```python
from build123d import *

# Parameters (mm, degrees)
SKETCH_1_W             = 49.2
SKETCH_1_H             = 40
EXTRUDE_1_DEPTH        = 8
HOLE_WIZARD_M4_1_D     = 3.3
HOLE_WIZARD_M4_1_DEPTH = 10.1
HOLE_WIZARD_M4_1_TIP   = 0.991420021
CHAMFER_1_SIZE         = 2
SKETCH_8_W             = 55.272888483
SKETCH_8_H             = 36.198084545
CUT_EXTRUDE_3_DEPTH    = 2
SKETCH_9_R             = 4.25
CUT_EXTRUDE_4_DEPTH    = 25
HOLE_WIZARD_M4_2_D     = 3.3
HOLE_WIZARD_M4_2_DEPTH = 10.1
HOLE_WIZARD_M4_2_TIP   = 0.991420021


with BuildPart() as part:
    # 草图1 → 凸台-拉伸1 (new body)
    with BuildSketch(Plane.XY):
        Rectangle(SKETCH_1_W, SKETCH_1_H)
    extrude(amount=EXTRUDE_1_DEPTH)

    # M4 螺纹孔1
    with Locations(Plane(origin=(0, -20, 0), x_dir=(-1, 0, 0), z_dir=(0, -1, 0))):
        with Locations((12.7, -4), (-12.7, -4)):
            Hole(HOLE_WIZARD_M4_1_D / 2, depth=HOLE_WIZARD_M4_1_DEPTH)
            with Locations((0, 0, -(HOLE_WIZARD_M4_1_DEPTH + HOLE_WIZARD_M4_1_TIP / 2))):  # 118° drill point
                Cone(0, HOLE_WIZARD_M4_1_D / 2, HOLE_WIZARD_M4_1_TIP, mode=Mode.SUBTRACT)

    # 倒角1
    chamfer_1_edges = [part.edges().sort_by_distance(p)[0] for p in [
        (-24.6, 20, 4),
        (24.6, 20, 4),
    ]]
    chamfer(chamfer_1_edges, length=CHAMFER_1_SIZE)

    # 草图8 → 切除-拉伸3 (cut)
    with BuildSketch(Plane.XY.offset(8)):
        with Locations((2.667874568, 4.099042273)):
            Rectangle(SKETCH_8_W, SKETCH_8_H)
    extrude(amount=-CUT_EXTRUDE_3_DEPTH, mode=Mode.SUBTRACT)

    # 草图9 → 切除-拉伸4 (cut)
    with BuildSketch(Plane(origin=(0, 0, 0), x_dir=(-1, 0, 0), z_dir=(0, 0, -1))):
        with Locations((-15, 6)):
            Circle(SKETCH_9_R)
        with Locations((15, 6)):
            Circle(SKETCH_9_R)
    extrude(amount=-CUT_EXTRUDE_4_DEPTH, mode=Mode.SUBTRACT)

    # M4 螺纹孔2
    with Locations(Plane.XY.offset(6)):
        with Locations((0, -4)):
            Hole(HOLE_WIZARD_M4_2_D / 2, depth=HOLE_WIZARD_M4_2_DEPTH)
            with Locations((0, 0, -(HOLE_WIZARD_M4_2_DEPTH + HOLE_WIZARD_M4_2_TIP / 2))):  # 118° drill point
                Cone(0, HOLE_WIZARD_M4_2_D / 2, HOLE_WIZARD_M4_2_TIP, mode=Mode.SUBTRACT)


solid = part.part
```
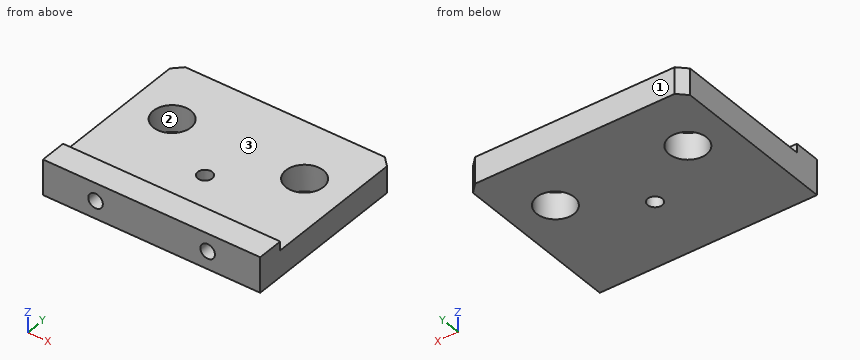
Can you work these out from the model? Positions are in its coordinate system, mm. Face numbers are marked on the shaded views. Coordinates: 2 decimals unless noted, no trailing zeros. Loops run counter-clockwise (first coordinate to the right, second up) from the corner with the lowest first, then second, coordinate; pieces in that order, holes last. Notation, with made-up numbers: (-39.75, 57) -> (-34.75, 57) arc R23 ccw to (-34.75, 87) -> close; hole circle Ø2 at (0.25, 13.5). An arc over 180 degrees is marked (long way). Answer as a JSON object with one key per item and string values.
1) Imagine slicing it at B-B (y = -4). Please give me the cut outline in (x, z).
Results:
{"outline": "(-24.6, 0) -> (-1.65, 0) -> (-1.65, 6) -> (-24.6, 6) -> close; (1.65, 0) -> (24.6, 0) -> (24.6, 6) -> (1.65, 6) -> close"}
2) Imagine slicing it at A-A (z = 1.5). Please give me the cut outline in (x, y).
Results:
{"outline": "(-24.6, -20) -> (24.6, -20) -> (24.6, 18) -> (22.6, 20) -> (-22.6, 20) -> (-24.6, 18) -> close; hole circle Ø8.5 at (-15, 6); hole circle Ø3.3 at (0, -4); hole circle Ø8.5 at (15, 6)"}
3) Imagine slicing it at C-C (x = 0). Please give me the cut outline in (y, z).
Results:
{"outline": "(-20, 0) -> (-5.65, 0) -> (-5.65, 6) -> (-14, 6) -> (-14, 8) -> (-20, 8) -> close; (-2.35, 0) -> (20, 0) -> (20, 6) -> (-2.35, 6) -> close"}
4) If I drill on line 1 (X direction, y = -16.75, z = 4); line 2 (Z direction, x = 12.7, y = -12.25); line 3 (X direction, y = -16.5, z = 2.75), over which ranges is the centre line in solid material (lowest first)?
Results:
{"line 1": "x = -24.6 to -14.35, -11.05 to 11.05, 14.35 to 24.6", "line 2": "z = 0 to 2.35, 5.65 to 6", "line 3": "x = -24.6 to -13.78, -11.62 to 11.62, 13.78 to 24.6"}
5) For P1, Ø3, axis at x = 12.7, z = 4, coming from the -Y side; P2, Ø10, axis at x = 8.5, y = 6.5, coming from the +Z side; P3, Ø0.6, axis at x = -5, z = 7, coming from the +Y side; P4, Ø12, axis at x = -7, y = 0.5, coming from the -Z side, each with a flat end and sliding along its axis, tell me the tip position at first contact or that it passes through.
Results:
{"P1": "stops at y = -9.81", "P2": "stops at z = 6", "P3": "stops at y = -14", "P4": "stops at z = 0"}
6) Thinking about a two-plate mould opening in Y: for the marked faces 1, 2 and 3, which applies, pulls with the +Y half, pulls with the -Y half, needs draft (parallel to the pull), parting line crosses it, or undercut?
Results:
{"face 1": "pulls with the +Y half", "face 2": "undercut", "face 3": "needs draft"}
7) Imagine slicing it at D-D (y = -16). Please give me the cut outline in (x, z), then the cut area to 3 significant figures.
Results:
{"outline": "(-24.6, 0) -> (24.6, 0) -> (24.6, 8) -> (-24.6, 8) -> close; hole circle Ø3.3 at (-12.7, 4); hole circle Ø3.3 at (12.7, 4)", "area": "376 mm^2"}
